Verification items for the finished model (mm, model axes). Give positions to 0.01 mm unless a question says otherwise; leave off trailing zeros. Loops run counter-clockwise (first coordinate to the right, second up) from the corner with the lowest first, then second, coordinate; pieces in that order, holes last. Notation, with made-up numbers: M -16.75,56 L -1.75,56 A19 ccw -1.75,92 Z; hole C 64,-20.5 d1. An arc over 180 degrees is marked long. Answer in a Markdown table with one row per item.
```python
from build123d import *

# Parameters (mm, degrees)
BOSS_EXTRUDE1_DEPTH     = 12.5
CUT_EXTRUDE1_DEPTH      = 698.543905428
CUT_EXTRUDE1_DEPTH_BACK = 698.543905428
SKETCH2_R               = 66.5
FILLET1_R               = 700
CHAMFER1_SIZE           = 12
CHAMFER2_SIZE           = 12


with BuildPart() as part:
    # Sketch1 → Boss-Extrude1 (new, symmetric)
    with BuildSketch(Plane(origin=(0, 0, 0), x_dir=(0, 0, -1), z_dir=(1, 0, 0))):
        with BuildLine():
            Line((623, -1.2), (252.997154134, -1.2))
            ThreePointArc((252.997154134, -1.2), (0, -253), (-252.997154134, -1.2))
            Line((-252.997154134, -1.2), (-623, -1.2))
            Line((-623, -1.2), (-546.789689993, -242.561510288))
            ThreePointArc((-546.789689993, -242.561510288), (-510.001069598, -293.866486715), (-450, -313.5))
            Line((-450, -313.5), (360.949185183, -313.5))
            Line((360.949185183, -313.5), (623, -1.2))
        make_face()
    extrude(amount=BOSS_EXTRUDE1_DEPTH, both=True)

    # Sketch2 → Cut-Extrude1 (cut, two sides: drawn at the far end of the back side and taken through both)
    with BuildSketch(Plane(origin=(0, 0, 0), x_dir=(0, 0, -1), z_dir=(1, 0, 0)).offset(-CUT_EXTRUDE1_DEPTH_BACK)):
        with Locations((-450, -212)):
            Circle(SKETCH2_R)
    extrude(amount=CUT_EXTRUDE1_DEPTH + CUT_EXTRUDE1_DEPTH_BACK, mode=Mode.SUBTRACT)

    # Fillet1
    fillet1_edges = [part.edges().sort_by_distance(p)[0] for p in [
        (0, -313.5, -360.949185183),
    ]]
    fillet(fillet1_edges, radius=FILLET1_R)

    # Chamfer1
    chamfer1_edges = [part.edges().sort_by_distance(p)[0] for p in [
        (-12.5, -212, 516.5),
        (-12.5, -253, 0),
    ]]
    chamfer(chamfer1_edges, length=CHAMFER1_SIZE)

    # Chamfer2
    chamfer2_edges = [part.edges().sort_by_distance(p)[0] for p in [
        (12.5, -1.2, -437.998577067),
        (12.5, -1.2, 437.998577067),
    ]]
    chamfer(chamfer2_edges, length=CHAMFER2_SIZE)


solid = part.part
```
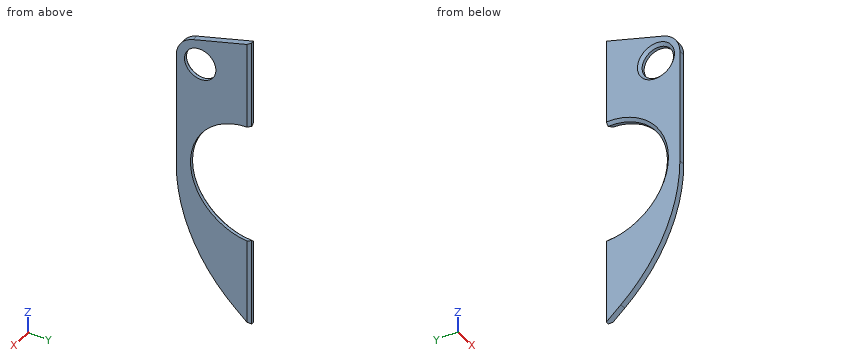
Item 1: Sectioned sample at B-B (z = 0). Record the cut outline in (x, y).
Reported:
| item | result |
|---|---|
| outline | M -12.5,-313.5 L 12.5,-313.5 L 12.5,-253 L -0.5,-253 L -12.5,-265 Z |
Item 2: Sectioned sample at C-C (y = -212). State how many separate pieces and enclosed holes the cut face has, and give its area (3 significant figures).
Reported:
| item | result |
|---|---|
| separate pieces | 3 |
| enclosed holes | 0 |
| area | 13,200 mm^2 |
Item 3: Scan lines: L1, parallel to Z at x = 3.5, y = -212; L2, parallel to Z at x = -7.25, y = -186; L3, parallel to Y at x = 9.75, z = 450. Record each from-to range of solid material in increasing order. Write a range as [from, to].
Reported:
| item | result |
|---|---|
| L1 | z = [-397.57, -138.08], [138.08, 383.5], [516.5, 556.44] |
| L2 | z = [-437.33, -181.31], [181.31, 381.52], [518.48, 564.65] |
| L3 | y = [-313.5, -278.5], [-145.5, -10.45] |
Item 4: Go/stop test with flat-tipped pins: pin 1 (10 mm diameter, centred on x = 6, z = -63.5, fed in from +Y); pin 2 (1 mm diameter, centred on x = -8, y = -121, fed in from +Z); pin 3 (2 mm diameter, centred on x = -9.5, y = -138, fed in from +Z). Record where each tip stops, or that it passes through.
Reported:
| item | result |
|---|---|
| pin 1 | stops at y = -243.55 |
| pin 2 | stops at z = 585.33 |
| pin 3 | stops at z = 580.12 |
Item 5: Sectioned sample at D-D (z = -441). Record the cut outline in (x, y).
Reported:
| item | result |
|---|---|
| outline | M -12.5,-183.4 L 12.5,-183.4 L 12.5,-13.2 L 0.5,-1.2 L -12.5,-1.2 Z |
